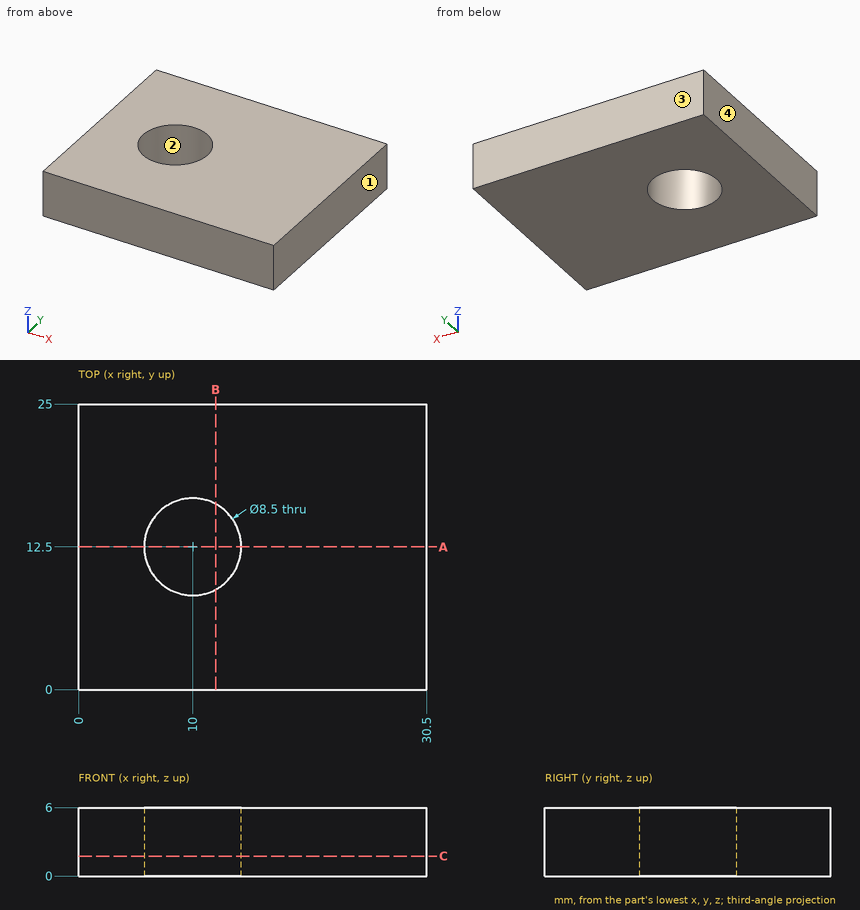
Could you check a few things on this drawing? It's one solid part, dimensions in mm from its lowest x, y, z. Give positions to 0.01 mm unless a question says otherwise; leave off trailing zeros. Loops run counter-clockwise (first coordinate to the right, second up) from the corner with the lowest first, then second, coordinate; pieces in that order, holes last. Notation, with made-up numbers: (57, 17) -> (66, 17) arc R24 cw to (66, 39) -> close; hole circle Ø9 at (-15, 63). An arc over 180 degrees is marked (long way). Use one line per item in the form item = value. Start each with the question number.
1) Thinking about a two-plate mould opening in X: for the marked faces 1, 2, 3 and 4, which applies, +X half, -X half, draft (parallel to the pull), parting line (faces both ways), or undercut?
2) Imagine slicing it at B-B (x = 12). Please give me the cut outline in (y, z).
3) Imagine slicing it at A-A (y = 12.5). Please give me the cut outline in (x, z).
4) Imagine slicing it at C-C (z = 1.75). Please give me the cut outline in (x, y), then the cut area to 3 significant figures.
5) Please list where these lines run through material, in increasing order: line 1 along Y through (x, z) = (10, 4.05); line 2 along Y through (x, z) = (8.5, 2.85); line 3 along X through (y, z) = (16.25, 5.6).
Check values:
q1.face_1 = +X half
q1.face_2 = undercut
q1.face_3 = draft
q1.face_4 = -X half
q2.outline = (0, 0) -> (8.75, 0) -> (8.75, 6) -> (0, 6) -> close; (16.25, 0) -> (25, 0) -> (25, 6) -> (16.25, 6) -> close
q3.outline = (0, 0) -> (5.75, 0) -> (5.75, 6) -> (0, 6) -> close; (14.25, 0) -> (30.5, 0) -> (30.5, 6) -> (14.25, 6) -> close
q4.outline = (0, 0) -> (30.5, 0) -> (30.5, 25) -> (0, 25) -> close; hole circle Ø8.5 at (10, 12.5)
q4.area = 706 mm^2
q5.line_1 = 0 to 8.25, 16.75 to 25
q5.line_2 = 0 to 8.52, 16.48 to 25
q5.line_3 = 0 to 8, 12 to 30.5
